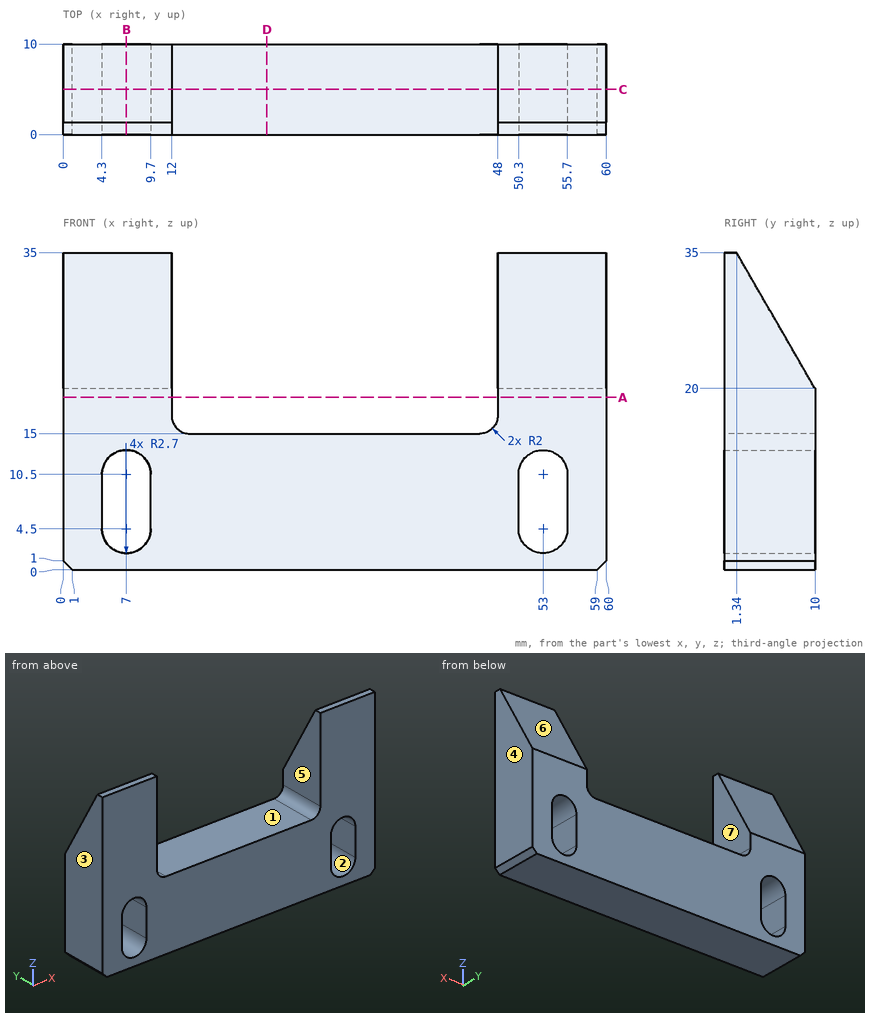
Check sheet for the drawn part. Datum: minimum x, y, z corner. Units: mm. A direction names the side the tool comes from. Round coordinates to 2 decimals unless told otherwise and drop trailing zeros. Write each loop counter-clockwise with the first axis right and the second up, starting at its lowest first coordinate (ties: lowest second). Pieces come first, ordered by that corner, then holes. Notation, with made-up numbers: (62, -20) - (96, -20) arc R21 cw to (96, 17) - close; hole circle Ø8 at (48.25, -3). An arc over 180 degrees is marked (long way). Return JSON: item names as keys, results as strings.
Q1. Access from +Z, -Z, +X, -X, +Y, -Y to the whole of each face (thin tool, end or side, straight path). Record for the marked faces 1, 2 and 3.
Returned:
{"face 1": "+Z, +Y, -Y", "face 2": "+Y, -Y", "face 3": "+Z, -Z, -X, +Y, -Y"}
Q2. Draft check along X on the marked faces 4, 5, 6 and 7. Enter one of: released by +X, released by -X, zero draft, split by the parting line, or undercut.
Returned:
{"face 4": "released by +X", "face 5": "undercut", "face 6": "zero draft", "face 7": "undercut"}
Q3. Cross-section at D-D (x = 22.5). Record the boundary of the cut face in (y, z).
Returned:
{"outline": "(0, 0) - (10, 0) - (10, 15) - (0, 15) - close"}
Q4. Depth check by flat-ended pin: P1, Ø4, axis at x = 41, y = 6.5, coming from the -Z side; P2, Ø6, axis at x = 7, z = 24.5, coming from the +Y side. Enter the tip coordinate at first touch or a pass-through.
Returned:
{"P1": "stops at z = 0", "P2": "stops at y = 9.13"}
Q5. Scan lines: L1, parallel to X at y = 1.5, z = 8.5; L2, parallel to X at y = 7.75, z = 22; L3, parallel to Z at x = 16.5, y = 6. Record each from-to range of solid material in increasing order. Write a range as from..to.
Returned:
{"L1": "x = 0..4.3, 9.7..50.3, 55.7..60", "L2": "x = 0..12, 48..60", "L3": "z = 0..15"}
Q6. Cross-section at B-B (x = 7). Record the boundary of the cut face in (y, z).
Returned:
{"outline": "(0, 0) - (10, 0) - (10, 1.8) - (0, 1.8) - close; (0, 13.2) - (10, 13.2) - (10, 20) - (1.34, 35) - (0, 35) - close"}
Q7. Cross-section at A-A (z = 19). Record the boundary of the cut face in (x, y).
Returned:
{"outline": "(0, 0) - (12, 0) - (12, 10) - (0, 10) - close; (48, 0) - (60, 0) - (60, 10) - (48, 10) - close"}
Q8. Cross-section at C-C (y = 5). Record the boundary of the cut face in (x, z), then the cut area to 3 significant figures.
Returned:
{"outline": "(0, 1) - (1, 0) - (59, 0) - (60, 1) - (60, 28.66) - (48, 28.66) - (48, 17) arc R2 cw to (46, 15) - (14, 15) arc R2 cw to (12, 17) - (12, 28.66) - (0, 28.66) - close; hole (4.3, 4.5) arc R2.7 ccw to (9.7, 4.5) - (9.7, 10.5) arc R2.7 ccw to (4.3, 10.5) - close; hole (50.3, 4.5) arc R2.7 ccw to (55.7, 4.5) - (55.7, 10.5) arc R2.7 ccw to (50.3, 10.5) - close", "area": "1,120 mm²"}
